Verification items for the finished model (mm, model axes). Face numbers are marked on the shaded views. Round coordinates to 2 decimals unless told otherwise and drop trailing zeros. Order: outer loops, then holes, each group sorted by start corner. A loop starts at its lowest first (then second) coordinate and runs counter-clockwise, first axis right, second up. Notation, with made-up numbers: M 17.25,82.25 L 57.25,82.25 A29 cw 57.25,110.25 Z; hole C 74.5,-18.75 d7. An arc over 180 degrees is marked long. Use one line per item in the form item = value. Start each with the question number.
Item 1: Cross-section at B-B on y = 113.5. Enter the section's corners in (x, z), then the cut area to 3 significant figures.
Item 2: Release check for a two-part mould opening along Y. For the marked faces 1 and 2 record: +Y half, -Y half, draft (parallel to the pull), parting line (faces both ways), or undercut.
Item 3: Thickness scan on probe 1 along Y at (x, z) = (0, 0.75); probe 2 along Y at (x, z) = (-5.5, -2.25); probe 3 along Y at (x, z) = (-2.25, 1.25). Record the ranges inside material, lowest first. Write a range as [from, to].
Item 4: Cross-section at A-A on x = 0. Enter the section's corners in (y, z), then the cut area to 3 significant figures.
Item 5: Go/stop test with flat-tipped pins: pin 1 Ø3.5 at (y, z) = (-2, 0) entering from -X; pin 2 Ø3.5 at (y, z) = (-3, 0) entering from +X; pin 3 Ø5 at (x, y) = (0, -6) entering from +Z. Record where each tip stops, or that it passes through.
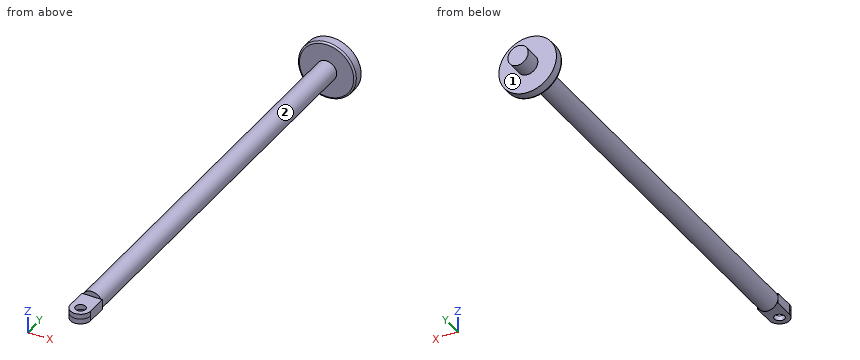
from build123d import *

# Parameters (mm, degrees)
SKETCH1_R           = 3
BOSS_EXTRUDE1_DEPTH = 130
SKETCH2_R           = 3
SKETCH2_R_2         = 1.5
BOSS_EXTRUDE2_DEPTH = 1.5
SKETCH3_R           = 8.5
BOSS_EXTRUDE3_DEPTH = 3
FILLET1_R           = 0.5


with BuildPart() as part:
    # Sketch1 → Boss-Extrude1 (new body)
    with BuildSketch(Plane(origin=(0, 0, 0), x_dir=(1, 0, 0), z_dir=(0, 1, 0))):
        with Locations(Location((0, 0, 0), (0, 0, 270))):
            Circle(SKETCH1_R)
    extrude(amount=BOSS_EXTRUDE1_DEPTH)

    # Sketch2 → Boss-Extrude2 (add, symmetric)
    # profile 1 of 2: a face of its own
    with BuildSketch(Plane.XY):
        with BuildLine():
            Line((3, 0), (-3, 0))
            Line((-3, 0), (-3, -6))
            ThreePointArc((-3, -6), (0, -3), (3, -6))
            Line((3, -6), (3, 0))
        make_face()
    # profile 2 of 2: a face of its own
    with BuildSketch(Plane.XY):
        with Locations((0, -6)):
            Circle(SKETCH2_R)
        with Locations((0, -6)):
            Circle(SKETCH2_R_2, mode=Mode.SUBTRACT)
    extrude(amount=BOSS_EXTRUDE2_DEPTH, both=True)

    # Sketch3 → Boss-Extrude3 (add)
    with BuildSketch(Plane(origin=(0, 122, 0), x_dir=(1, 0, 0), z_dir=(0, 1, 0))):
        with Locations(Location((0, 0, 0), (0, 0, 270))):
            Circle(SKETCH3_R)
    extrude(amount=BOSS_EXTRUDE3_DEPTH)

    # Fillet1
    fillet1_edges = [part.edges().sort_by_distance(p)[0] for p in [
        (0, 122, -8.5),
    ]]
    fillet(fillet1_edges, radius=FILLET1_R)


solid = part.part
Output values:
q1.outline = C 0,0 d6
q1.area = 28.3 mm2
q2.face_1 = +Y half
q2.face_2 = undercut
q3.probe_1 = [-9, -7.5], [-4.5, 130]
q3.probe_2 = [122, 125]
q3.probe_3 = [-7.98, 130]
q4.outline = M -9,-1.5 L -7.5,-1.5 L -7.5,1.5 L -9,1.5 Z; M -4.5,-1.5 L 0,-1.5 L 0,-3 L 122,-3 L 122,-8 A0.5 ccw 122.5,-8.5 L 125,-8.5 L 125,-3 L 130,-3 L 130,3 L 125,3 L 125,8.5 L 122.5,8.5 A0.5 ccw 122,8 L 122,3 L 0,3 L 0,1.5 L -4.5,1.5 Z
q4.area = 831 mm2
q5.pin_1 = -3
q5.pin_2 = 3
q5.pin_3 = 1.5
